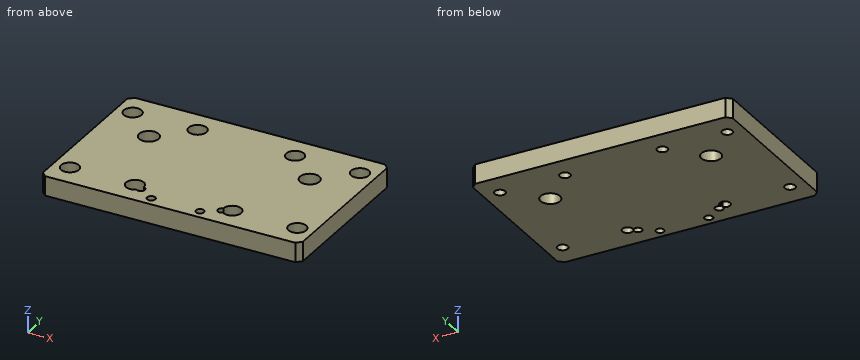
```python
from build123d import *

# Parameters (mm, degrees)
SKETCH_1_W                   = 160
SKETCH_1_H                   = 100
EXTRUDE_1_DEPTH              = 12
HOLE_WIZARD_M14_1_D          = 12
HOLE_WIZARD_M6_1_D           = 6.4
HOLE_WIZARD_M6_1_CBORE_D     = 11
HOLE_WIZARD_M6_1_CBORE_DEPTH = 6.4
CHAMFER_1_SIZE               = 3
HOLE_WIZARD_M6_1_2_D         = 5
HOLE_WIZARD_M6_2_D           = 5
HOLE_WIZARD_M6_2_DEPTH       = 15
HOLE_WIZARD_M6_2_TIP         = 1.502151548


with BuildPart() as part:
    # 草图1 → 凸台-拉伸1 (new body)
    with BuildSketch(Plane.XY):
        with Locations((80, 50)):
            Rectangle(SKETCH_1_W, SKETCH_1_H)
    extrude(amount=EXTRUDE_1_DEPTH)

    # M14 螺纹孔1 (through all)
    with Locations(Plane.XY.offset(12)):
        with Locations((30.5, 66), (129.5, 66)):
            Hole(HOLE_WIZARD_M14_1_D / 2)

    # Hole Wizard M6 _1 (through all)
    with Locations(Plane.XY.offset(12)):
        with Locations((10, 15), (50, 15), (50, 85), (10, 85), (110, 15), (150, 15), (150, 85), (110, 85)):
            CounterBoreHole(HOLE_WIZARD_M6_1_D / 2, HOLE_WIZARD_M6_1_CBORE_D / 2, HOLE_WIZARD_M6_1_CBORE_DEPTH)

    # 倒角1
    chamfer_1_edges = [part.edges().sort_by_distance(p)[0] for p in [
        (0, 100, 6),
        (160, 100, 6),
        (160, 0, 6),
        (0, 0, 6),
    ]]
    chamfer(chamfer_1_edges, length=CHAMFER_1_SIZE)

    # Hole Wizard M6 _1 2 (through all)
    with Locations(Plane(origin=(0, 0, 0), x_dir=(-1, 0, 0), z_dir=(0, 0, -1))):
        with Locations((-65, 6), (-95, 6)):
            Hole(HOLE_WIZARD_M6_1_2_D / 2)

    # M6 螺纹孔2
    with Locations(Plane.XY.offset(12)):
        with Locations((55, 12.5), (105, 12.5)):
            Hole(HOLE_WIZARD_M6_2_D / 2, depth=HOLE_WIZARD_M6_2_DEPTH)
            with Locations((0, 0, -(HOLE_WIZARD_M6_2_DEPTH + HOLE_WIZARD_M6_2_TIP / 2))):  # 118° drill point
                Cone(0, HOLE_WIZARD_M6_2_D / 2, HOLE_WIZARD_M6_2_TIP, mode=Mode.SUBTRACT)


solid = part.part
```
Geometry: final body of the model. Coordinates: model frame, mm. Coordinates: 2 decimals unless noted, no trailing zeros. Order: outer loops, then holes, each group sorted by start corner. A loop starts at its lowest first (then second) coordinate and runs counter-clockwise, first axis right, second up. Notation, with made-up numbers: M 4.25,69 L 34.25,69 A12 cw 34.25,88 Z; hole C 32,-28.5 d6. An arc over 180 degrees is marked long. Answer as CSV lines item,"result".
Q1. Section A-A on x = 150. Return the cut outline in (y, z), and give its area (3 significant figures).
Answers:
outline,"M 0,0 L 11.8,0 L 11.8,5.6 L 9.5,5.6 L 9.5,12 L 0,12 Z; M 18.2,0 L 81.8,0 L 81.8,5.6 L 79.5,5.6 L 79.5,12 L 20.5,12 L 20.5,5.6 L 18.2,5.6 Z; M 88.2,0 L 100,0 L 100,12 L 90.5,12 L 90.5,5.6 L 88.2,5.6 Z"
area,"988 mm^2"
Q2. First-contact query: P1, Ø4, axis at x = 10, y = 85, coming from the -Z side; P2, Ø6.5, axis at x = 10, y = 15, coming from the +Z side. Flat tips, straight axial feed; report the tip coordinate or a pass-through.
Answers:
P1,"passes through"
P2,"stops at z = 5.6"
Q3. Line query: probe 1 along Y at (x, z) = (50, 7); probe 2 along Y at (x, z) = (129.5, 7.25); probe 3 along Y at (x, z) = (46.5, 11). Output: solid intervals per line, ascending. Write a range as [from, to].
Answers:
probe 1,"y = [0, 9.5], [20.5, 79.5], [90.5, 100]"
probe 2,"y = [0, 60], [72, 100]"
probe 3,"y = [0, 10.76], [19.24, 80.76], [89.24, 100]"
Q4. Section C-C on z = 3. Count the separate pieces of the cut face and the enclosed holes in it, and give its area (3 significant figures).
Answers:
separate pieces,"1"
enclosed holes,"12"
area,"15,400 mm^2"
Q5. Section B-B on x = 30.5. Return the cut outline in (y, z).
Answers:
outline,"M 0,0 L 60,0 L 60,12 L 0,12 Z; M 72,0 L 100,0 L 100,12 L 72,12 Z"
